The listing builds one solid part. Answer for the finished solid, in the listing's coordinates (mm). A direction names the side the tool comes from. Round coordinates to 2 decimals unless told otherwise and drop trailing zeros. Order: outer loops, then holes, each group sorted by start corner. A loop starts at its lowest first (then second) coordinate and runs counter-clockwise, first axis right, second up. Notation, with made-up numbers: (89.25, 80) - (122.25, 80) arc R28 ccw to (122.25, 100) - close; hole circle Ø8 at (88.5, 7.5). An arc over 180 degrees is marked (long way). One line per item, written item: value. Start each with the question number.
1. Section A-A, the plane z = -60 is taken. Give the vertices of the cut face in (x, y), then the cut area to 3 significant figures.
2. Section D-D, the plane x = -39 is taken. Give the vertices of the cut face in (y, z), then the cut area to 3 significant figures.
3. For a pull along X with two mould halves and no side action, classify faces 1 (the cylindrical face through (117.075, 62.082, 6.538)), 2 (the flat face through (15, 30, 2)), 3 (the flat face through (58, 50, 0)) as released by +X, released by -X, zero draft, split by the parting line, or undercut.
4. Straight lines are drawn through the part: line 1 (X direction, y = 54.5, z = 0); line 2 (Z direction, x = 0, y = 15); line 3 (X direction, y = -4.5, z = -60). For each, find the intervals that lie inside material, in ascending order.
5. Section C-C, the plane x = 74 is taken. Give the vertices of the cut face in (y, z).
6. A tool of negligible diameter and unlimited length cuts with its end or side. For faces 4 (the flat face through (107, 70, 1)), 5 (the cylindrical face through (-125.912, -2.082, -60.684)), 6 (the flat face through (15, 30, -2)), from which of +Z, -Z, +X, -X, +Y, -Y can it reach the whole face along a straight path? Write none if from no direction.
7. Section B-B, the plane x = 0 is taken. Give the vertices of the cut face in (y, z).
8. Flat-ended cylindrical pins translate along their axes: P1, Ø1.5, axis at x = 16, y = 15.5, coming from the +Z side; P2, Ø12, axis at y = 60.5, z = -25, coming from the -X side; P3, Ø10, axis at y = 46.5, z = -11.5, coming from the +X side. Find the tip coordinate at first contact, or state that the pin passes through.
from build123d import *

# Parameters (mm, degrees)
HUB_PROFILE_SKETCH_R       = 31
HUB_62_KEYED_BORE_26_DEPTH = 50
ARM_A_PLATE_DEPTH          = 10
SKETCH2_4_R                = 20.281835497
SKETCH2_4_R_2              = 7.37420564
ARM_A_END_BOSS_DEPTH       = 20
ARM_B_PLATE_DEPTH          = 10
ARM_B_END_BOSS_DEPTH       = 10
ARM_B_END_BOSS_DEPTH_BACK  = 10
SKETCH4_3_R                = 22
SKETCH4_3_R_2              = 7.5


with BuildPart() as part:
    # Hub Profile Sketch → Hub _62 Keyed Bore _26 (new body)
    with BuildSketch(Plane(origin=(0, 0, 0), x_dir=(1, 0, 0), z_dir=(0, 1, 0))):
        with Locations(Location((0, 0, 0), (0, 0, 270))):
            Circle(HUB_PROFILE_SKETCH_R)
        with BuildLine():
            Line((12.845232579, -2), (18, -2))
            Line((18, -2), (18, 2))
            Line((18, 2), (12.845232579, 2))
            ThreePointArc((12.845232579, 2), (-13, 0), (12.845232579, -2))
        make_face(mode=Mode.SUBTRACT)
    extrude(amount=HUB_62_KEYED_BORE_26_DEPTH)

    # Arm A Sketch → Arm A Plate (add)
    with BuildSketch(Plane(origin=(0, 50, 0), x_dir=(1, 0, 0), z_dir=(0, 1, 0))):
        with BuildLine():
            ThreePointArc((3.394741403, 30.813564072), (-31, 0), (3.394741403, -30.813564072))
            Line((3.394741403, -30.813564072), (100.096839243, -20.159859277))
            ThreePointArc((100.096839243, -20.159859277), (77.593984821, 0), (100.096839243, 20.159859277))
            Line((100.096839243, 20.159859277), (3.394741403, 30.813564072))
        make_face()
        with BuildLine():
            Line((18, 2), (18, 0))
            Line((18, 0), (18, -2))
            Line((18, -2), (12.845232579, -2))
            ThreePointArc((12.845232579, -2), (-13, 0), (12.845232579, 2))
            Line((12.845232579, 2), (18, 2))
        make_face(mode=Mode.SUBTRACT)
    extrude(amount=ARM_A_PLATE_DEPTH)

    # Sketch2_4 → Arm A End Boss (add)
    with BuildSketch(Plane(origin=(0, 50, 0), x_dir=(1, 0, 0), z_dir=(0, 1, 0))):
        with Locations(Location((97.875820318, 0, 0), (0, 0, 83.713057555))):
            Circle(SKETCH2_4_R)
        with Locations(Location((97.875820318, 0, 0), (0, 0, 270))):
            Circle(SKETCH2_4_R_2, mode=Mode.SUBTRACT)
    extrude(amount=ARM_A_END_BOSS_DEPTH)

    # Arm B Sketch → Arm B Plate (add)
    with BuildSketch(Plane.XZ):
        with BuildLine():
            Line((-17.469853837, 25.608674447), (-116.321009242, -41.826102006))
            ThreePointArc((-116.321009242, -41.826102006), (-93.645771026, -40.54807031), (-81.923048454, -60))
            ThreePointArc((-81.923048454, -60), (-85.296700275, -71.70722655), (-94.382971499, -79.823897994))
            Line((-94.382971499, -79.823897994), (13.442835709, -27.933674447))
            ThreePointArc((13.442835709, -27.933674447), (-26.846787517, -15.5), (-17.469853837, 25.608674447))
        make_face()
    extrude(amount=-ARM_B_PLATE_DEPTH)

    # Sketch4_3 → Arm B End Boss (add, two sides: drawn at the far end of the back side and taken through both)
    with BuildSketch(Plane.XZ.offset(-ARM_B_END_BOSS_DEPTH_BACK)):
        with Locations(Location((-103.923048454, -60, 0), (0, 0, 124.301222305))):
            Circle(SKETCH4_3_R)
        with Locations(Location((-103.923048454, -60, 0), (0, 0, 270))):
            Circle(SKETCH4_3_R_2, mode=Mode.SUBTRACT)
    extrude(amount=ARM_B_END_BOSS_DEPTH + ARM_B_END_BOSS_DEPTH_BACK)


solid = part.part
Answer list:
1. outline: (-125.92, -10) - (-111.42, -10) - (-111.42, 10) - (-125.92, 10) - close; (-96.42, -10) - (-81.92, -10) - (-81.92, 0) - (-53.19, 0) - (-53.19, 10) - (-96.42, 10) - close
1. area: 867 mm²
2. outline: (0, -53.17) - (10, -53.17) - (10, 10.92) - (0, 10.92) - close
2. area: 641 mm²
3. face 1: split by the parting line
3. face 2: undercut
3. face 3: zero draft
4. line 1: x = -31 to -13, 18 to 90.5, 105.25 to 118.16
4. line 2: z = -31 to -13, 13 to 31
4. line 3: x = -125.92 to -111.42, -96.42 to -81.92
5. outline: (50, -23.03) - (60, -23.03) - (60, 23.03) - (50, 23.03) - close
6. face 4: +Z, -Z, +X, -X, +Y
6. face 5: -Y
6. face 6: +Y, -Y
7. outline: (0, -34.4) - (10, -34.4) - (10, -31) - (60, -31) - (60, -13) - (0, -13) - close; (0, 13) - (60, 13) - (60, 31) - (0, 31) - close
8. P1: stops at z = 26.99
8. P2: stops at x = -24.48
8. P3: stops at x = 116.54
